Model file for the job. Use its own axes, mm. A direction names the side the tool comes from. Round coordinates to 2 decimals unless told otherwise and drop trailing zeros. Order: outer loops, then holes, each group sorted by start corner. A loop starts at its lowest first (then second) coordinate and runs counter-clockwise, first axis right, second up. Notation, with made-up numbers: (13.25, -5) -> (51.25, -5) arc R19 cw to (51.25, 18) -> close; hole circle Ø7 at (-9.75, 57). An arc over 180 degrees is marked (long way). Put each result on its own line as item: value. Start each with the question number.
Q1. 3-axis set-ups, long thin cutter, end or side, ignore diameter. For faces 5 (the face through (-118.914, 26.622, 44.122)), 6 (the face through (-78.552, 47.902, -30.431)), 7 (the face through (101.527, 20.787, 22.545)), 8 (the face through (-134, 27, -42.5)), 9 (the face through (-122, 10, 0)): which of +Z, -Z, +X, -X, +Y, -Y reach the whole face in a straight line?
Q2. Pull direction Z, two halves, no side cores. Call faces 1 (the face through (-85.51, 27.88, -85.25)), 2 (the face through (124.908, 26.622, 4.798)), 3 (the face through (-154, 27, 0)), 4 (the face through (-142.853, 44.987, 32.351)): released by +Z, released by -Z, zero draft, split by the parting line, or undercut.
Q3. Cut at B-B, the plane y = 45.5. State how many separate pieces and enclosed holes the cut face has, and give its area (3 significant figures).
Q4. Probe L1, parallel to Z at x = -106, y = 52; L2, parallel to Z at x = -146.25, y = 48.5; L3, parallel to X at y = 46.5, z = 32.5. List the from-to ranges inside material, lowest first.
Q5. Flat gauge pins, fed straight in: P1, Ø12, axis at x = 23.5, y = 13.5, coming from the -Z side; P2, Ø5, axis at x = 62, z = 33.5, coming from the -Y side; P3, Ø1.5, axis at y = 40, z = -54.5, coming from the +X side. Where does each tip first touch, or does it go through?
Q6. Cut at A-A, the plane x = 0. List the corners of the cut face in (y, z), and give its area (3 significant figures).
from build123d import *

# Parameters (mm, degrees)
SKETCH_3_W             = 50
SKETCH_3_H             = 85
EXTRUDE_1_DEPTH        = 55
SKETCH_5_R             = 31.25
CUT_EXTRUDE_1_DEPTH    = 45
HOLE_WIZARD_M8_1_D     = 6.8
HOLE_WIZARD_M8_1_DEPTH = 19.75
HOLE_WIZARD_M8_1_TIP   = 2.042926105
FILLET_1_R             = 10
HOLE_WIZARD_M10_1_D    = 8.5
CHAMFER_1_SIZE         = 1


with BuildPart() as part:
    # 草图2 → 旋转1 (revolve)
    with BuildSketch(Plane.XY, mode=Mode.PRIVATE) as revolve_1_sk:
        Polygon((104, 0), (104, 41), (50, 41), (50, 50), (48, 50), (48, 55), (125, 55), (125, 0), align=None)
    revolve(revolve_1_sk.sketch.rotate(Axis((0, 0, 0), (0, 1, 0)), 90), axis=Axis((0, 0, 0), (0, 1, 0)))

    # 草图3 → 凸台-拉伸1 (add, through all)
    with BuildSketch(Plane(origin=(0, 55, 0), x_dir=(1, 0, 0), z_dir=(0, 1, 0))):
        with Locations((-129, 0)):
            Rectangle(SKETCH_3_W, SKETCH_3_H)
    extrude(amount=-EXTRUDE_1_DEPTH)

    # 草图5 → 切除-拉伸1 (cut)
    with BuildSketch(Plane(origin=(0, 55, 0), x_dir=(1, 0, 0), z_dir=(0, 1, 0))):
        with Locations(Location((-113.75, 0, 0), (0, 0, 270))):
            Circle(SKETCH_5_R)
    extrude(amount=-CUT_EXTRUDE_1_DEPTH, mode=Mode.SUBTRACT)

    # M8 螺纹孔1
    with Locations(Plane(origin=(0, 55, 0), x_dir=(1, 0, 0), z_dir=(0, 1, 0))):
        with Locations((-146.25, 32.5), (-113.75, 0), (-81.25, 32.5), (-146.25, -32.5), (-81.25, -32.5)):
            Hole(HOLE_WIZARD_M8_1_D / 2, depth=HOLE_WIZARD_M8_1_DEPTH)
            with Locations((0, 0, -(HOLE_WIZARD_M8_1_DEPTH + HOLE_WIZARD_M8_1_TIP / 2))):  # 118° drill point
                Cone(0, HOLE_WIZARD_M8_1_D / 2, HOLE_WIZARD_M8_1_TIP, mode=Mode.SUBTRACT)

    # 圆角1
    fillet_1_edges = [part.edges().sort_by_distance(p)[0] for p in [
        (-117.553179455, 27.5, 42.5),
        (-117.553179455, 27.5, -42.5),
        (-154, 27.5, 42.5),
        (-154, 27.5, -42.5),
    ]]
    fillet(fillet_1_edges, radius=FILLET_1_R)

    # M10 螺纹孔1 (through all)
    with Locations(Plane(origin=(0, 0, 0), x_dir=(-1, 0, 0), z_dir=(0, -1, 0))):
        with Locations((-107.631965538, -44.582619871), (-107.631965538, 44.582619871), (-44.582619871, 107.631965538), (44.582619871, 107.631965538), (107.631965538, 44.582619871), (107.631965538, -44.582619871), (44.582619871, -107.631965538), (-44.582619871, -107.631965538), (0, 116.5), (-82.377940008, 82.377940008), (82.377940008, 82.377940008), (-82.377940008, -82.377940008), (82.377940008, -82.377940008), (-116.5, 0)):
            Hole(HOLE_WIZARD_M10_1_D / 2)

    # 倒角1
    chamfer_1_edges = [part.edges().sort_by_distance(p)[0] for p in [
        (-154, 55, 0),
        (125, 55, 0),
        (-134.186714819, 55, -42.5),
        (-134.186714819, 55, 42.5),
        (-151.071067812, 55, -39.571067812),
        (-151.071067812, 55, 39.571067812),
        (-118.845721654, 55, -44.166666667),
        (-118.845721654, 55, 44.166666667),
    ]]
    chamfer(chamfer_1_edges, length=CHAMFER_1_SIZE)


solid = part.part
Ans:
1. face 5: +Z, -X, +Y, -Y
1. face 6: +Y, -Y
1. face 7: -Y
1. face 8: -Z, -X, +Y, -Y
1. face 9: +Y
2. face 1: undercut
2. face 2: split by the parting line
2. face 3: zero draft
2. face 4: undercut
3. separate pieces: 1
3. enclosed holes: 20
3. area: 39,900 mm^2
4. L1: z = -66.25 to -48.51, -40.66 to -30.27, 30.27 to 40.66, 48.51 to 66.25
4. L2: z = -42.24 to -35.9, -29.1 to 29.1, 35.9 to 42.24
4. L3: x = -154 to -149.65, -142.85 to -84.65, -77.85 to -38, 38 to 120.7
5. P1: stops at z = -123.77
5. P2: stops at y = 41
5. P3: stops at x = 112.85
6. outline: (0, -125) -> (54, -125) -> (55, -124) -> (55, -120.75) -> (0, -120.75) -> close; (0, -112.25) -> (55, -112.25) -> (55, -48) -> (50, -48) -> (50, -50) -> (41, -50) -> (41, -104) -> (0, -104) -> close; (0, 104) -> (41, 104) -> (41, 50) -> (50, 50) -> (50, 48) -> (55, 48) -> (55, 124) -> (54, 125) -> (0, 125) -> close
6. area: 3,370 mm^2
